Verification items for the finished model (mm, model axes). A direction names the side the tool comes from. Round coordinates to 2 decimals unless told otherwise and drop trailing zeros. Order: outer loops, then holes, each group sorted by start corner. A loop starts at its lowest first (then second) coordinate and runs counter-clockwise, first axis right, second up. Notation, with made-up numbers: M 79,53 L 125,53 A13 ccw 125,71 Z; hole C 54.5,31.25 d8. An arc over 180 degrees is marked long. Use CSV: the item, a comma, the result in double quotes. Start each with the question number.
Q1. Sectioned sample at B-B (x = 31). Enter the section's corners in (y, z).
Q2. Mould release check, pull along Z, two halves, no side actions. Record for faces 3 (the face through (1, 6, -12.5)), 4 (the face through (-27.005, 8.874, 2.28)), 5 (the face through (-37, 18, 0)): +Z half, -Z half, draft (parallel to the pull), parting line (faces both ways), or undercut.
Q3. Scan lines: line 1 (X direction, y = 15.5, z = -2.75); line 2 (X direction, y = 2, z = 4.75); line 3 (X direction, y = 8, z = 4.5). Record each from-to range of solid material in increasing order.
Q4. Gauge pin test, flat ends, axial feed: pin 1 Ø6 at (y, z) = (20, -10) entering from +X; pin 2 Ø13 at (x, z) = (-32, 2.5) entering from +Y; pin 3 Ø8 at (x, z) = (31, 3.5) entering from +Y; pin 4 Ø5 at (y, z) = (24, 6.5) entering from +X. Record the tip position at first contact, or that the pin passes through.
Q5. Sectioned sample at A-A (y = 16). Enter the section's corners in (x, z), and give its area (3 significant figures).
Q6. Set-up check for faces 1 (the face through (36, 18, 0)), 2 (the face through (35.995, 8.874, 3.28)): record each of +Z, -Z, +X, -X, +Y, -Y from which the full face is reachable in a straight line by a thin tool's end or side.
Q7. Sectioned sample at D-D (z = -9.5). Enter the section's corners in (x, y).
Q8. Sectioned sample at C-C (z = 3.5). Enter the section's corners in (x, y), and give its area (3 significant figures).
```python
from build123d import *

# Parameters (mm, degrees)
PILLOW_BLOCK_PROFILE_R  = 9
PILLOW_BLOCK_BODY_DEPTH = 12.5
MOUNTING_HOLES_2X_10_D  = 10


with BuildPart() as part:
    # Pillow Block Profile → Pillow Block Body (new, symmetric)
    with BuildSketch(Plane.XY):
        with BuildLine():
            Line((46, 0), (-46, 0))
            Line((-46, 0), (-46, 18))
            Line((-46, 18), (-22, 18))
            ThreePointArc((-22, 18), (-16.727922061, 30.727922061), (-4, 36))
            Line((-4, 36), (4, 36))
            ThreePointArc((4, 36), (16.727922061, 30.727922061), (22, 18))
            Line((22, 18), (46, 18))
            Line((46, 18), (46, 0))
        make_face()
        with Locations((0, 16)):
            Circle(PILLOW_BLOCK_PROFILE_R, mode=Mode.SUBTRACT)
    extrude(amount=PILLOW_BLOCK_BODY_DEPTH, both=True)

    # Mounting Holes 2xØ10 (through all)
    with Locations(Plane(origin=(-32, 18, 2.5), x_dir=(1, 0, 0), z_dir=(0, 1, 0))):
        with Locations((0, 0), (63, -1)):
            Hole(MOUNTING_HOLES_2X_10_D / 2)


solid = part.part
```
Verdict:
1,outline,"M 0,-12.5 L 18,-12.5 L 18,-1.5 L 0,-1.5 Z; M 0,8.5 L 18,8.5 L 18,12.5 L 0,12.5 Z"
2,face 3,"-Z half"
2,face 4,"undercut"
2,face 5,"draft"
3,line 1,"x = -46 to -8.99, 8.99 to 46"
3,line 2,"x = -46 to -36.47, -27.53 to 26.16, 35.84 to 46"
3,line 3,"x = -46 to -36.58, -27.42 to -4.12, 4.12 to 26.1, 35.9 to 46"
4,pin 1,"stops at x = 46"
4,pin 2,"stops at y = 18"
4,pin 3,"passes through"
4,pin 4,"stops at x = 21.66"
5,outline,"M -46,-12.5 L -9,-12.5 L -9,12.5 L -46,12.5 Z; M 9,-12.5 L 46,-12.5 L 46,12.5 L 9,12.5 Z; hole C -32,2.5 d10; hole C 31,3.5 d10"
5,area,"1,690 mm²"
6,face 1,"+Z, -Z, +X, +Y"
6,face 2,"+Y, -Y"
7,outline,"M -46,0 L 46,0 L 46,18 L 22,18 A18 ccw 4,36 L -4,36 A18 ccw -22,18 L -46,18 Z; hole C 0,16 d18"
8,outline,"M -46,0 L -36.9,0 L -36.9,18 L -46,18 Z; M -27.1,0 L 26,0 L 26,18 L 22,18 A18 ccw 4,36 L -4,36 A18 ccw -22,18 L -27.1,18 Z; M 36,0 L 46,0 L 46,18 L 36,18 Z; hole C 0,16 d18"
8,area,"1,700 mm²"
